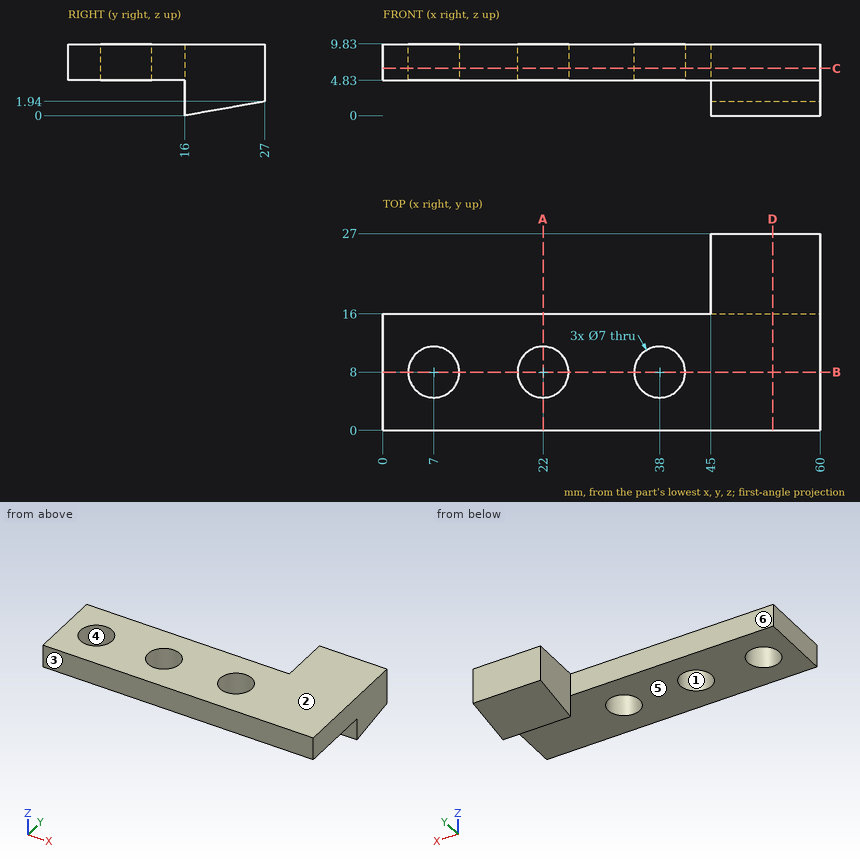
The figure shows three views and two pictorial views of one solid part (mm, origin at its lowest corner). Answer the questions. A direction names the side the tool comes from. Give positions to 0.01 mm unless a question says otherwise; leave off trailing zeros. Loops run counter-clockwise (first coordinate to the right, second up) from the corner with the lowest first, then second, coordinate; pieces in that order, holes last. Notation, with made-up numbers: (-16.5, 89.25) -> (11.5, 89.25) arc R24 cw to (11.5, 116.25) -> close; hole circle Ø8 at (-26, -26). An arc over 180 degrees is marked (long way). Use a Markdown table: item, result. Add a question column.
1. For the marked faces 4, 5 and 6, determine the directions among +Z, -Z, +X, -X, +Y, -Y from which every point of the face is accessible in a straight line to the end or side of a thin tool.
2. Determine the mould class of the marked faces 1, 2 and 3 for opening direction Y: released by +Y, released by -Y, zero draft, split by the parting line, or undercut.
3. Section B-B on y = 8 is taken. Determine the outline of the cut face in (x, z).
4. Section C-C on z = 6.5 is taken. Determine the outline of the cut face in (x, y).
5. Section A-A on x = 22 is taken. Determine the outline of the cut face in (y, z).
6. Flat-ended cylindrical pins translate along their axes: pin 1 Ø1.5 at (x, y) = (29, 16) entering from -Z; pin 2 Ø1 at (y, z) = (8, 3) entering from +X; pin 3 Ø4 at (x, z) = (56, 2) entering from -Y; pin 4 Ø5.5 at (x, z) = (18.5, 7) entering from +Y. Find the tip coordinate at first contact, or state that the pin passes through.
7. Section D-D on x = 53.5 is taken. Determine the outline of the cut face in (y, z).
8. Find the intervals of material crossed by probe 1 along X at (y, z) = (9.25, 8); probe 2 along Y at (x, z) = (22, 8.5); probe 3 along X at (y, z) = (10, 6.5), in increasing order.
Results below:
| question | item | result |
|---|---|---|
| 1 | face 4 | +Z, -Z |
| 1 | face 5 | -Z, +X, -X, -Y |
| 1 | face 6 | +Z, -Z, -X, +Y |
| 2 | face 1 | undercut |
| 2 | face 2 | zero draft |
| 2 | face 3 | released by -Y |
| 3 | outline | (0, 4.83) -> (3.5, 4.83) -> (3.5, 9.83) -> (0, 9.83) -> close; (10.5, 4.83) -> (18.5, 4.83) -> (18.5, 9.83) -> (10.5, 9.83) -> close; (25.5, 4.83) -> (34.5, 4.83) -> (34.5, 9.83) -> (25.5, 9.83) -> close; (41.5, 4.83) -> (60, 4.83) -> (60, 9.83) -> (41.5, 9.83) -> close |
| 4 | outline | (0, 0) -> (60, 0) -> (60, 27) -> (45, 27) -> (45, 16) -> (0, 16) -> close; hole circle Ø7 at (7, 8); hole circle Ø7 at (22, 8); hole circle Ø7 at (38, 8) |
| 5 | outline | (0, 4.83) -> (4.5, 4.83) -> (4.5, 9.83) -> (0, 9.83) -> close; (11.5, 4.83) -> (16, 4.83) -> (16, 9.83) -> (11.5, 9.83) -> close |
| 6 | pin 1 | stops at z = 4.83 |
| 6 | pin 2 | passes through |
| 6 | pin 3 | stops at y = 16 |
| 6 | pin 4 | stops at y = 16 |
| 7 | outline | (0, 4.83) -> (16, 4.83) -> (16, 0) -> (27, 1.94) -> (27, 9.83) -> (0, 9.83) -> close |
| 8 | probe 1 | x = 0 to 3.73, 10.27 to 18.73, 25.27 to 34.73, 41.27 to 60 |
| 8 | probe 2 | y = 0 to 4.5, 11.5 to 16 |
| 8 | probe 3 | x = 0 to 4.13, 9.87 to 19.13, 24.87 to 35.13, 40.87 to 60 |
